Work out the finished part from the listing and answer in its coordinate system (mm). Face numbers are marked on the shaded views. A direction names the side the tool comes from. Round coordinates to 2 decimals unless told otherwise and drop trailing zeros. Write each loop counter-clockwise with the first axis right and the second up, starting at its lowest first coordinate (ties: lowest second). Pieces come first, ordered by that corner, then holes. Notation, with made-up numbers: (-32, 49) -> (-18, 49) arc R21 cw to (-18, 75) -> close; hole circle Ø9 at (82.25, 10). An arc over 180 degrees is marked (long way). One line per question, with ' | ' between items. Start each with the question number.
```python
from build123d import *

# Parameters (mm, degrees)
SKETCH4_W          = 1.383873909
SKETCH4_H          = 8
CUT_EXTRUDE1_DEPTH = 5


with BuildPart() as part:
    # Sketch1 → Revolve1 (revolve)
    with BuildSketch(Plane.XY, mode=Mode.PRIVATE) as revolve1_sk:
        Polygon((0, 0), (4.3, 0), (4.8, 0.5), (4.8, 11.5), (4.3, 12), (0, 12), align=None)
    revolve(revolve1_sk.sketch.rotate(Axis((0, 12, 0), (0, 1, 0)), 90), axis=Axis((0, 12, 0), (0, 1, 0)))

    # Sketch3 → M5 Tapped Hole1 (revolve, cut)
    with BuildSketch(Plane(origin=(0, 12, 0), x_dir=(0, 0, 1), z_dir=(1, 0, 0))):
        Polygon((0, 0), (0, 12), (2.6, 12), (2.1, 11.5), (2.1, 0.5), (2.6, 0), align=None)
    revolve(axis=Axis((0, 18.35, 0), (0, -1, 0)), mode=Mode.SUBTRACT)

    # Sketch4 → Cut-Extrude1 (cut, symmetric)
    with BuildSketch(Plane.XY):
        with Locations((-4.641936955, 8)):
            Rectangle(SKETCH4_W, SKETCH4_H)
        with Locations((4.641936955, 8)):
            Rectangle(SKETCH4_W, SKETCH4_H)
    extrude(amount=CUT_EXTRUDE1_DEPTH, both=True, mode=Mode.SUBTRACT)


solid = part.part
```
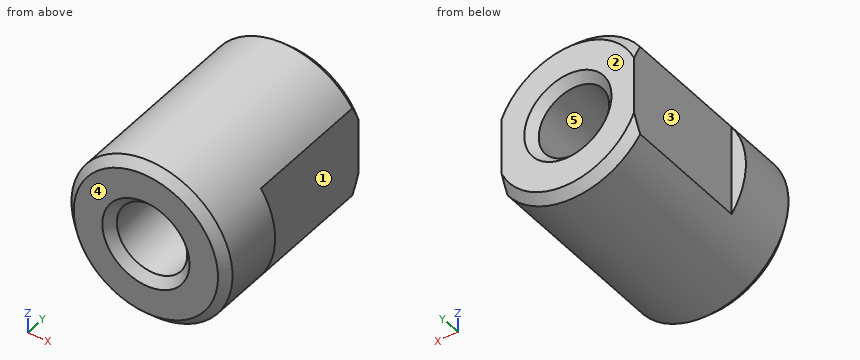
(1) A cutting plane is placed at C-C, the plane z = 0. Determine the outline of the cut face in (x, y).
(2) The mould has two halves that part along X. Classify the marked faces 3, 4 and 5: +X half, -X half, draft (parallel to the pull), parting line (faces both ways), or undercut.
(3) For the marked faces 1 and 2, determine the directions among +Z, -Z, +X, -X, +Y, -Y from which every point of the face is accessible in a straight line to the end or side of a thin tool.
(4) Consider L1, parallel to X at y = 3, z = 0; L2, parallel to X at y = 6.25, z = 0; L3, parallel to Z at x = 4.25, y = 2.5. Determine where each line is inside the solid, lowest interval first.
(5) Given pin 1 Ø4 at (y, z) = (10.5, 0.5) entering from +X; pin 2 Ø1 at (x, z) = (1, -1) entering from -Y; pin 3 Ø2.5 at (y, z) = (9, -1) entering from -X; pin 4 Ø3 at (x, y) = (-2.5, 9) entering from -Z, each flat-ended and moving along its own axis, determine where each tip first touches the part or whether it passes through.
(6) A cutting plane is placed at A-A, the plane x = 0. Determine the outline of the cut face in (y, z), then the cut area to 3 significant figures.
(7) A cutting plane is placed at B-B, the plane y = 10.5. Determine the outline of the cut face in (x, z).
Returned:
1) outline: (-4.8, 0.5) -> (-4.3, 0) -> (-2.6, 0) -> (-2.1, 0.5) -> (-2.1, 11.5) -> (-2.6, 12) -> (-3.95, 12) -> (-3.95, 4) -> (-4.8, 4) -> close; (2.1, 0.5) -> (2.6, 0) -> (4.3, 0) -> (4.8, 0.5) -> (4.8, 4) -> (3.95, 4) -> (3.95, 12) -> (2.6, 12) -> (2.1, 11.5) -> close
2) face 3: -X half | face 4: draft | face 5: undercut
3) face 1: +Z, -Z, +X, +Y | face 2: +Z, -Z, +X, -X, +Y
4) L1: -4.8 to -2.1, 2.1 to 4.8 | L2: -3.95 to -2.1, 2.1 to 3.95 | L3: -2.23 to 2.23
5) pin 1: x = 3.95 | pin 2: through | pin 3: x = -3.95 | pin 4: z = -4.69
6) outline: (0, -4.3) -> (0.5, -4.8) -> (11.5, -4.8) -> (12, -4.3) -> (12, -2.6) -> (11.5, -2.1) -> (0.5, -2.1) -> (0, -2.6) -> close; (0, 2.6) -> (0.5, 2.1) -> (11.5, 2.1) -> (12, 2.6) -> (12, 4.3) -> (11.5, 4.8) -> (0.5, 4.8) -> (0, 4.3) -> close | area: 63.8 mm2
7) outline: (-3.95, -2.73) arc R4.8 ccw to (3.95, -2.73) -> (3.95, 2.73) arc R4.8 ccw to (-3.95, 2.73) -> close; hole circle Ø4.2 at (0, 0)
